```python
from build123d import *

# Parameters (mm, degrees)
SKETCH1_R           = 15
SKETCH1_R_2         = 9.5
BOSS_EXTRUDE1_DEPTH = 9
CUT_EXTRUDE1_START  = 6
SKETCH2_R           = 10
SKETCH2_R_2         = 9.5
CUT_EXTRUDE1_DEPTH  = 1.1
CHAMFER1_SIZE       = 0.5


with BuildPart() as part:
    # Sketch1 → Boss-Extrude1 (new, symmetric)
    with BuildSketch(Plane.XY):
        Circle(SKETCH1_R)
        Circle(SKETCH1_R_2, mode=Mode.SUBTRACT)
    extrude(amount=BOSS_EXTRUDE1_DEPTH, both=True)

    # Sketch2 → Cut-Extrude1 (cut)
    with BuildSketch(Plane.XY.offset(CUT_EXTRUDE1_START)):
        Circle(SKETCH2_R)
        Circle(SKETCH2_R_2, mode=Mode.SUBTRACT)
    cut_extrude1 = extrude(amount=CUT_EXTRUDE1_DEPTH, mode=Mode.SUBTRACT)

    # Mirror1: Cut-Extrude1 across plane
    add(cut_extrude1.mirror(Plane.XY), mode=Mode.SUBTRACT)

    # Chamfer1
    chamfer1_edges = [part.edges().sort_by_distance(p)[0] for p in [
        (-15, 0, -9),
        (-15, 0, 9),
        (-9.5, 0, -9),
        (-9.5, 0, 9),
    ]]
    chamfer(chamfer1_edges, length=CHAMFER1_SIZE)


solid = part.part
```
The model under review builds one solid part; all positions refer to its coordinate system, in mm. A direction names the side the tool comes from. Coordinates: 2 decimals unless noted, no trailing zeros. Write each loop counter-clockwise with the first axis right and the second up, starting at its lowest first coordinate (ties: lowest second). Pieces come first, ordered by that corner, then holes. Notation, with made-up numbers: (54, 14) - (101, 14) arc R21 cw to (101, 24) - close; hole circle Ø9 at (-38.75, 51). An arc over 180 degrees is marked (long way). Answer in a Markdown table with one row per item. Add a question column.
Q1. To check wall thickness, follow line 1 along Y through (x, z) = (0, -8); line 2 along Y through (x, z) = (0, 6.7); line 3 along Z through (x, y) = (-5.5, -8). State the ranges of each line that lie inside material, in increasing order. Write a range as from..to.
Q2. Consider section C-C on z = 2.75. Give the boundary of the cut face in (x, y), then the cut area to 3 significant figures.
Q3. Draft analysis for pull direction Y (two halves, no side actions). For faces 1 (the face through (-14.985, 0.66, 0.119)), 2 (the face through (3, 10, 9)), 3 (the face through (4.38, -8.43, -7.81)), state which applies: +Y half, -Y half, draft (parallel to the pull), parting line (faces both ways), or undercut.
Q4. Clearance check with flat-ended pins moving along their axes: pin 1 (10 mm diameter, centred on y = -8.5, z = -6.5, fed in from -X); pin 2 (2 mm diameter, centred on x = 5.5, z = 1, fed in from +Y); pin 3 (5 mm diameter, centred on x = 8.5, z = 4.5, fed in from +Y). State where each tip first meets the part, or that it passes through.
Q5. For faces 4 (the face through (3, 10, -9)), 5 (the face through (-2.17, -9.76, 6.54)), list the 3-axis set-ups (+Z, -Z, +X, -X, +Y, -Y) from which the entire face can be reached by the end or side of a thin tool; tool diameter is ignored.
Answers below:
| question | item | result |
|---|---|---|
| 1 | line 1 | -15..-9.5, 9.5..15 |
| 1 | line 2 | -15..-10, 10..15 |
| 1 | line 3 | -8.71..-7.1, -6..6, 7.1..8.71 |
| 2 | outline | circle Ø30 at (0, 0); hole circle Ø19 at (0, 0) |
| 2 | area | 423 mm² |
| 3 | face 1 | parting line |
| 3 | face 2 | draft |
| 3 | face 3 | undercut |
| 4 | pin 1 | x = -14.59 |
| 4 | pin 2 | y = 14.31 |
| 4 | pin 3 | y = 13.75 |
| 5 | face 4 | -Z, +X, -X, +Y, -Y |
| 5 | face 5 | none |
